Design review of the part built by this model. Coordinates are the model's own, in mm. Coordinates: 2 decimals unless noted, no trailing zeros. Write each loop counter-clockwise with the first axis right and the second up, starting at its lowest first coordinate (ties: lowest second). Pieces come first, ordered by that corner, then holes. Notation, with made-up numbers: M 3.25,-31 L 27.25,-31 A13 cw 27.25,-26 Z; hole C 81,31 d1. An arc over 180 degrees is marked long. Return JSON: item names as keys, results as strings. Group by question number.
```python
from build123d import *

# Parameters (mm, degrees)
SKETCH1_R           = 2
BOSS_EXTRUDE1_DEPTH = 3


with BuildPart() as part:
    # Sketch1 → Boss-Extrude1 (new body)
    with BuildSketch(Plane.XY):
        Polygon((10, 0), (170, 0), (180, -10), (180, -100), (170, -110), (10, -110), (0, -100), (0, -10), align=None)
        with Locations((90, -10)):
            Circle(SKETCH1_R, mode=Mode.SUBTRACT)
        with Locations((117.5, -10)):
            Circle(SKETCH1_R, mode=Mode.SUBTRACT)
        with Locations((62.5, -10)):
            Circle(SKETCH1_R, mode=Mode.SUBTRACT)
    extrude(amount=BOSS_EXTRUDE1_DEPTH)


solid = part.part
```
Item 1: For pin 1 (5 mm diameter, centred on x = 161.5, y = -17.5, fed in from -Z), flat-tipped, find the tip position at first contact; note if it passes through.
Item 2: The part is to be moulded in two halves that separate along Y. For faces 1 (the cylindrical face through (91.908, -9.399, 1.479)), 2 (the cylindrical face through (61.026, -8.648, 1.479)), 3 (the flat face through (5, -5, 1)), 4 (the flat face through (91, -54, 3)), say which applies: pulls with the +Y half, pulls with the -Y half, needs draft (parallel to the pull), parting line crosses it, or undercut.
Item 3: For line 1 (Y direction, x = 117.5, z = 2.35); line 2 (X direction, y = -9.5, z = 2.45); line 3 (X direction, y = -11, z = 1.25), list the stretches that pass through material, from the lowest coordinate up.
Item 4: Add section A-A (x = 117.5). Write out the cut boundary in (y, z), plus the area to 3 significant figures.
Geometry check:
{
 "1": {"pin 1": "z = 0"},
 "2": {"face 1": "undercut", "face 2": "undercut", "face 3": "pulls with the +Y half", "face 4": "needs draft"},
 "3": {"line 1": "-110 to -12, -8 to 0", "line 2": "0.5 to 60.56, 64.44 to 88.06, 91.94 to 115.56, 119.44 to 179.5", "line 3": "0 to 60.77, 64.23 to 88.27, 91.73 to 115.77, 119.23 to 180"},
 "4": {"outline": "M -110,0 L -12,0 L -12,3 L -110,3 Z; M -8,0 L 0,0 L 0,3 L -8,3 Z", "area": "318 mm^2"}
}
